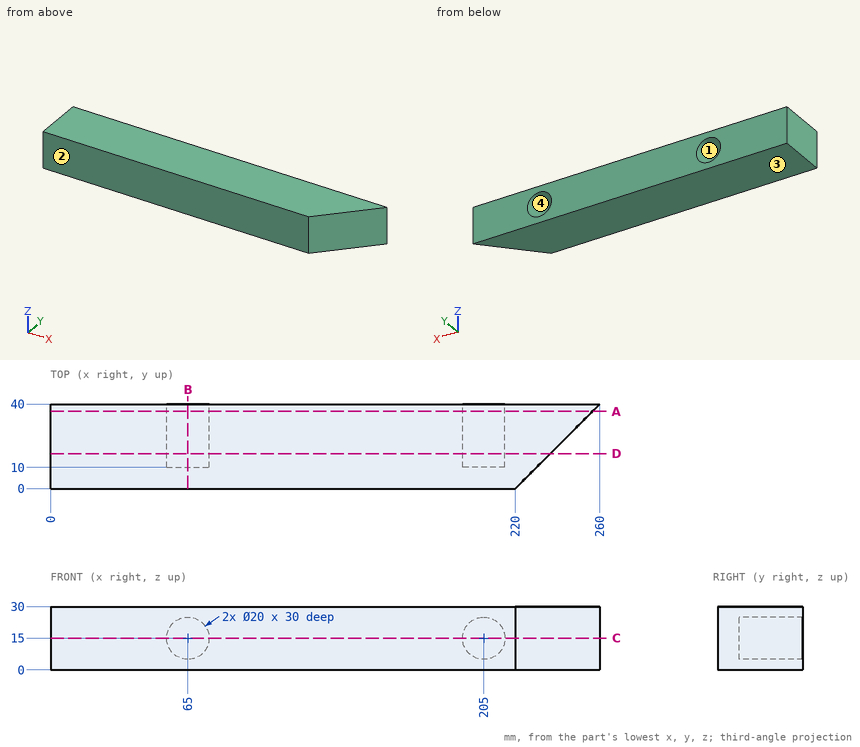
Input: dimensioned drawing with shaded views. Units: mm. Origin: part minimum x, y, z. Give positions to 0.01 mm unless a question says otherwise; leave off trailing zeros. Write each loop counter-clockwise with the first axis right and the second up, starting at its lowest first coordinate (ties: lowest second). Pieces come first, ordered by that corner, then holes. Notation, with made-up numbers: M 14,-14 L 71,-14 A28 ccw 71,5 Z; hole C 30,19 d10. An arc over 180 degrees is marked long. Return JSON: item names as keys, results as strings. Group by question number.
1) Pull-direction query (Z, two-part tool) for the marked faces 1, 2, 3 and 4; classes: pulls with the +Z half, pulls with the -Z half, needs draft (parallel to the pull), parting line crosses it, or undercut.
2) Cut plane C-C, the plane z = 15. Output: boundary loops of the cut face in (x, y).
3) Cut plane B-B, the plane x = 65. Output: boundary loops of the cut face in (y, z).
4) Material intervals for line 1 along X through (y, z) = (34, 21.5); line 2 along X through (y, z) = (25, 24); line 3 along Z through (x, y) = (65, 16), sorted ascending. Write a range as [from, to].
5) Cut plane D-D, the plane y = 16.5. Output: boundary loops of the cut face in (x, z).
6) Cut plane A-A, the plane y = 36.5. Output: boundary loops of the cut face in (x, z), plus the area to 3 significant figures.
7) Pin query (flat end, axial travel): P1, Ø8, axis at y = 30, z = 13.5, coming from the -X side; P2, Ø6, axis at x = 209, z = 19.5, coming from the +Y side. Return the tip coordinate at first contact, or that it passes through.
Recorded:
{
 "1": {"face 1": "undercut", "face 2": "needs draft", "face 3": "pulls with the -Z half", "face 4": "undercut"},
 "2": {"outline": "M 0,0 L 220,0 L 260,40 L 215,40 L 215,10 L 195,10 L 195,40 L 75,40 L 75,10 L 55,10 L 55,40 L 0,40 Z"},
 "3": {"outline": "M 0,0 L 40,0 L 40,5 L 10,5 L 10,25 L 40,25 L 40,30 L 0,30 Z"},
 "4": {"line 1": "x = [0, 57.4], [72.6, 197.4], [212.6, 254]", "line 2": "x = [0, 60.64], [69.36, 200.64], [209.36, 245]", "line 3": "z = [0, 5], [25, 30]"},
 "5": {"outline": "M 0,0 L 236.5,0 L 236.5,30 L 0,30 Z; hole C 65,15 d20; hole C 205,15 d20"},
 "6": {"outline": "M 0,0 L 256.5,0 L 256.5,30 L 0,30 Z; hole C 65,15 d20; hole C 205,15 d20", "area": "7,070 mm²"},
 "7": {"P1": "stops at x = 0", "P2": "stops at y = 10"}
}
